For this review, use the dimensioned drawing (mm, ordinates from the lowest corner) and the shaded views. Round coordinates to 2 decimals unless told otherwise and drop trailing zeros. Order: outer loops, then holes, each group sorted by start corner. A loop starts at its lowest first (then second) coordinate and runs counter-clockwise, first axis right, second up. Notation, with made-up numbers: M -24,37 L 7,37 A18 ccw 7,54 Z; hole C -13,35 d6. An arc over 180 degrees is marked long. One line per item, written item: value. Start each with the question number.
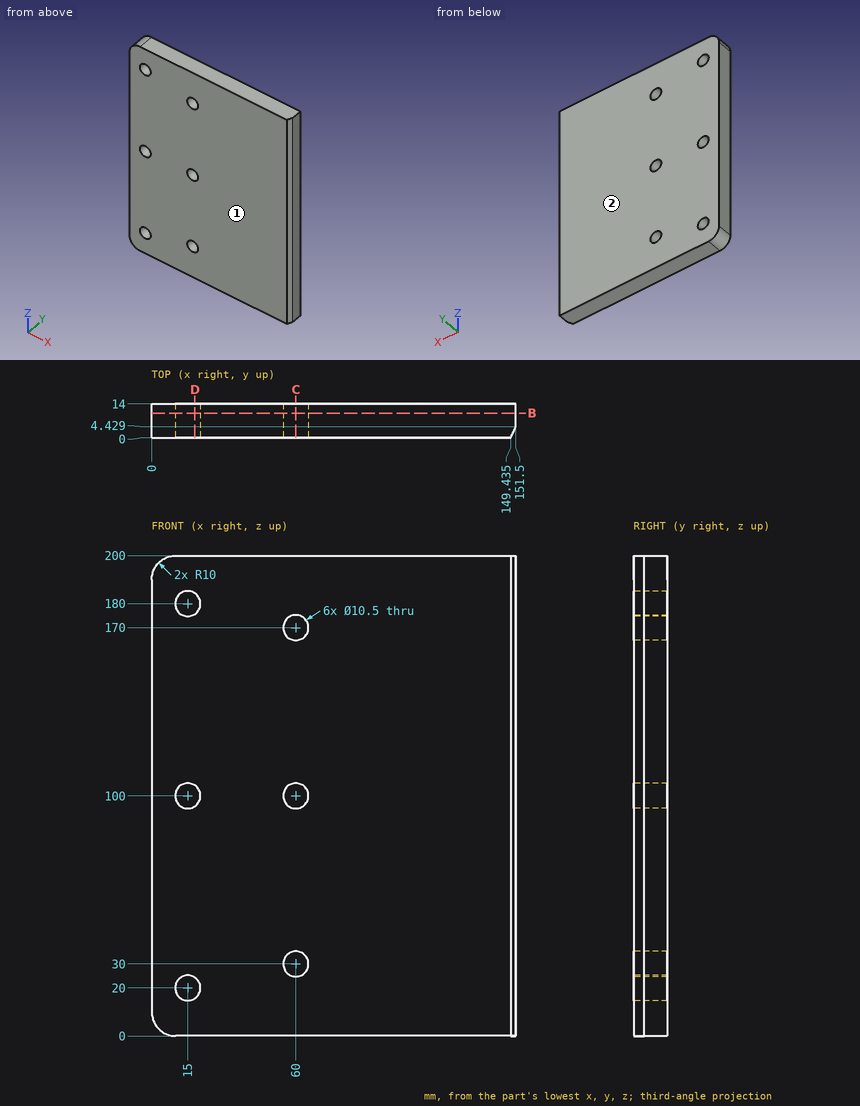
Item 1: Wall thickness on L1, parallel to Z at x = 15, y = 8.5; L2, parallel to Z at x = 60, y = 9.75; L3, parallel to X at y = 0.5, z = 172 (1 decimal): over which ranges is each line inside the solid? List them lowest first.
Item 2: Consider section B-B, the plane y = 10.25. Give the boundary of the cut face in (x, z).
Item 3: Clearance check with a flat-ended pin moving along its axis: P1, Ø9.5, axis at x = 15, z = 20, coming from the -Y side. State where the tip first meets the part, or that it passes through.
Item 4: Consider section D-D, the plane x = 18. Give the boundary of the cut face in (y, z), then the cut area to 3 significant figures.
Item 5: Consider section C-C, the plane x = 60. Give the boundary of the cut face in (y, z), then the cut area to 3 significant figures.
Item 6: The part is to be moulded in two halves that separate along Y. For the marked faces 1 and 2, say which applies: pulls with the +Y half, pulls with the -Y half, needs draft (parallel to the pull), parting line crosses it, or undercut.
Computed:
1. L1: z = 0 to 14.75, 25.25 to 94.75, 105.25 to 174.75, 185.25 to 200
1. L2: z = 0 to 24.75, 35.25 to 94.75, 105.25 to 164.75, 175.25 to 200
1. L3: x = 0 to 55.1, 64.9 to 149.7
2. outline: M 0,10 A10 ccw 10,0 L 151.5,0 L 151.5,200 L 10,200 A10 ccw 0,190 Z; hole C 15,20 d10.5; hole C 15,100 d10.5; hole C 15,180 d10.5; hole C 60,30 d10.5; hole C 60,100 d10.5; hole C 60,170 d10.5
3. P1: passes through
4. outline: M 0,0 L 14,0 L 14,15.69 L 0,15.69 Z; M 0,24.31 L 14,24.31 L 14,95.69 L 0,95.69 Z; M 0,104.31 L 14,104.31 L 14,175.69 L 0,175.69 Z; M 0,184.31 L 14,184.31 L 14,200 L 0,200 Z
4. area: 2,440 mm^2
5. outline: M 0,0 L 14,0 L 14,24.75 L 0,24.75 Z; M 0,35.25 L 14,35.25 L 14,94.75 L 0,94.75 Z; M 0,105.25 L 14,105.25 L 14,164.75 L 0,164.75 Z; M 0,175.25 L 14,175.25 L 14,200 L 0,200 Z
5. area: 2,360 mm^2
6. face 1: pulls with the -Y half
6. face 2: pulls with the +Y half
